Could you check a few things on this model? Use its own coordinates, in mm. Face numbers are marked on the shaded views. A direction names the side the tool comes from. Give positions to 0.01 mm unless a question says otherwise; leave off trailing zeros. Order: outer loops, then holes, each group sorted by start corner. A loop starts at its lowest first (then second) coordinate and runs counter-clockwise, first axis right, second up. Notation, with made-up numbers: (86.5, 59) -> (120.5, 59) arc R24 ccw to (120.5, 79) -> close; hole circle Ø8 at (85, 67). An arc over 180 degrees is marked (long way). Write each question's results on one line, items separated by ' | '.
```python
from build123d import *

# Parameters (mm, degrees)
SKETCH1_R           = 50
BOSS_EXTRUDE1_DEPTH = 20
SKETCH2_R           = 7.5
CUT_EXTRUDE1_DEPTH  = 15
SKETCH3_R           = 1
CUT_EXTRUDE2_DEPTH  = 74.484692283
SKETCH4_R           = 1.8
CUT_EXTRUDE3_DEPTH  = 4


with BuildPart() as part:
    # Sketch1 → Boss-Extrude1 (new body)
    with BuildSketch(Plane(origin=(0, 0, 0), x_dir=(1, 0, 0), z_dir=(0, 1, 0))):
        with Locations(Location((0, 0, 0), (0, 0, 270))):
            Circle(SKETCH1_R)
    extrude(amount=BOSS_EXTRUDE1_DEPTH)

    # Sketch2 → Cut-Extrude1 (cut)
    with BuildSketch(Plane(origin=(0, 20, 0), x_dir=(1, 0, 0), z_dir=(0, 1, 0))):
        with Locations(Location((0, 30, 0), (0, 0, 270))):
            Circle(SKETCH2_R)
        with Locations(Location((25.980762114, -15, 0), (0, 0, 270))):
            Circle(SKETCH2_R)
        with Locations(Location((-25.980762114, -15, 0), (0, 0, 270))):
            Circle(SKETCH2_R)
    extrude(amount=-CUT_EXTRUDE1_DEPTH, mode=Mode.SUBTRACT)

    # Sketch3 → Cut-Extrude2 (cut, through all)
    with BuildSketch(Plane.XZ):
        with Locations(Location((25.980762114, 19, 0), (0, 0, 270))):
            Circle(SKETCH3_R)
        with Locations(Location((29.980762114, 15, 0), (0, 0, 270))):
            Circle(SKETCH3_R)
        with Locations(Location((21.980762114, 15, 0), (0, 0, 270))):
            Circle(SKETCH3_R)
        with Locations(Location((25.980762114, 11, 0), (0, 0, 270))):
            Circle(SKETCH3_R)
        with Locations(Location((-25.980762114, 19, 0), (0, 0, 270))):
            Circle(SKETCH3_R)
        with Locations(Location((-29.980762114, 15, 0), (0, 0, 270))):
            Circle(SKETCH3_R)
        with Locations(Location((-25.980762114, 11, 0), (0, 0, 270))):
            Circle(SKETCH3_R)
        with Locations(Location((-21.980762114, 15, 0), (0, 0, 270))):
            Circle(SKETCH3_R)
        with Locations(Location((0, -26, 0), (0, 0, 270))):
            Circle(SKETCH3_R)
        with Locations(Location((-4, -30, 0), (0, 0, 270))):
            Circle(SKETCH3_R)
        with Locations(Location((0, -34, 0), (0, 0, 270))):
            Circle(SKETCH3_R)
        with Locations(Location((4, -30, 0), (0, 0, 270))):
            Circle(SKETCH3_R)
    extrude(amount=-CUT_EXTRUDE2_DEPTH, mode=Mode.SUBTRACT)

    # Sketch4 → Cut-Extrude3 (cut)
    with BuildSketch(Plane.XZ):
        with Locations(Location((-25.980762114, 19, 0), (0, 0, 270))):
            Circle(SKETCH4_R)
        with Locations(Location((-29.980762114, 15, 0), (0, 0, 270))):
            Circle(SKETCH4_R)
        with Locations(Location((-25.980762114, 11, 0), (0, 0, 270))):
            Circle(SKETCH4_R)
        with Locations(Location((-21.980762114, 15, 0), (0, 0, 270))):
            Circle(SKETCH4_R)
        with Locations(Location((25.980762114, 19, 0), (0, 0, 270))):
            Circle(SKETCH4_R)
        with Locations(Location((21.980762114, 15, 0), (0, 0, 270))):
            Circle(SKETCH4_R)
        with Locations(Location((25.980762114, 11, 0), (0, 0, 270))):
            Circle(SKETCH4_R)
        with Locations(Location((29.980762114, 15, 0), (0, 0, 270))):
            Circle(SKETCH4_R)
        with Locations(Location((0, -26, 0), (0, 0, 270))):
            Circle(SKETCH4_R)
        with Locations(Location((-4, -30, 0), (0, 0, 270))):
            Circle(SKETCH4_R)
        with Locations(Location((0, -34, 0), (0, 0, 270))):
            Circle(SKETCH4_R)
        with Locations(Location((4, -30, 0), (0, 0, 270))):
            Circle(SKETCH4_R)
    extrude(amount=-CUT_EXTRUDE3_DEPTH, mode=Mode.SUBTRACT)


solid = part.part
```
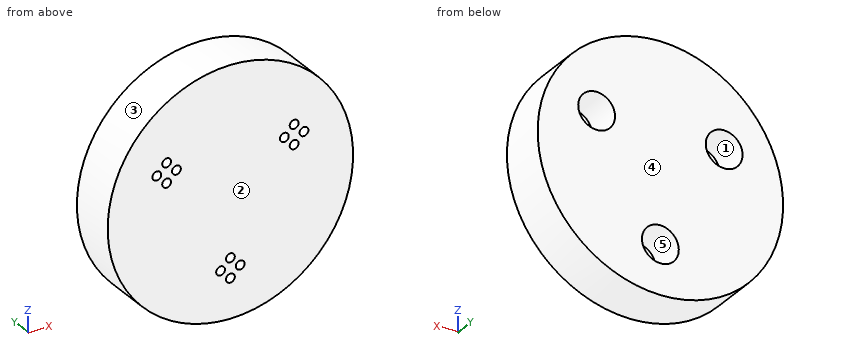
Q1. Suppose I cut it at A-A on y = 1.75. State how many separate pieces and enclosed holes the cut face has, and give its area (3 significant figures).
Here are the results:
separate pieces: 1 | enclosed holes: 12 | area: 7,730 mm²
Q2. I'm going to push flat-ended pins straight in: pin 1 Ø3 at (x, z) = (-26, 11.5) entering from -Y; pin 2 Ø1.8 at (x, z) = (-22.5, 15) entering from -Y; pin 3 Ø2 at (x, y) = (-10, 14) entering from +Z; pin 4 Ø4 at (x, z) = (-29.98, 15) entering from +Y. Where does each tip first touch, or does it pass through?
Here are the results:
pin 1: stops at y = 0 | pin 2: stops at y = 4 | pin 3: stops at z = 49.18 | pin 4: stops at y = 5
Q3. Suppose I cut it at C-C on y = 14.25. Please give me the cut outline in (x, z).
Here are the results:
outline: circle Ø100 at (0, 0); hole circle Ø15 at (-25.98, 15); hole circle Ø15 at (0, -30); hole circle Ø15 at (25.98, 15)
Q4. I need wall thicknesses on line 1 along X through (y, z) = (2.7, 15); line 2 along X through (y, z) = (1.15, 19); line 3 along X through (y, z) = (13.5, 15). Which ranges of each line are inside material? Lowest first, please.
Here are the results:
line 1: x = -47.7 to -31.78, -28.18 to -23.78, -20.18 to 20.18, 23.78 to 28.18, 31.78 to 47.7 | line 2: x = -46.25 to -27.78, -24.18 to 24.18, 27.78 to 46.25 | line 3: x = -47.7 to -33.48, -18.48 to 18.48, 33.48 to 47.7
Q5. Suppose I cut it at B-B on z = -40. Please give me the cut outline in (x, y), and give its area (3 significant figures).
Here are the results:
outline: (-30, 0) -> (30, 0) -> (30, 20) -> (-30, 20) -> close | area: 1,200 mm²
Q6. Thinking about a two-plate mould opening in Z: for the marked faces 1, 2 and 3, which applies, +Z half, -Z half, draft (parallel to the pull), parting line (faces both ways), or undercut?
Here are the results:
face 1: undercut | face 2: draft | face 3: parting line
Q7. Suppose I cut it at D-D on x = -42.5. Please give me the cut outline in (y, z).
Here are the results:
outline: (0, -26.34) -> (20, -26.34) -> (20, 26.34) -> (0, 26.34) -> close
Q8. For the marked faces 4 and 5, which set-ups out of +Z, -Z, +X, -X, +Y, -Y let a thin tool reach every point of the face, with its end or its side?
Here are the results:
face 4: +Z, -Z, +X, -X, +Y | face 5: +Y
